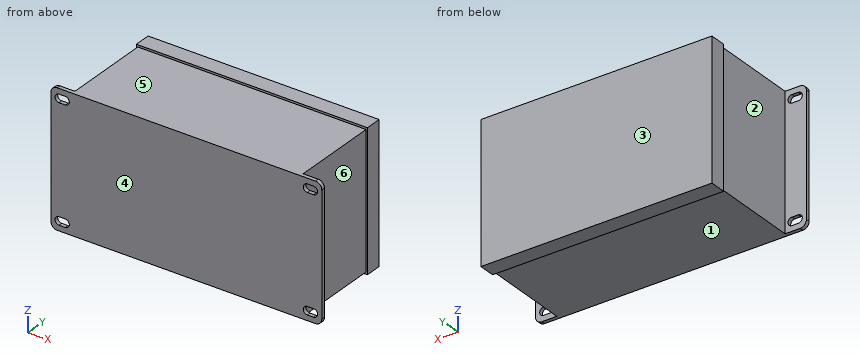
from build123d import *

# Parameters (mm, degrees)
BOSS_EXTRUDE1_DEPTH = 3
SKETCH2_W           = 182
SKETCH2_H           = 107
BOSS_EXTRUDE2_DEPTH = 70
SKETCH4_W           = 184.261814912
SKETCH4_H           = 110.411316032
BOSS_EXTRUDE3_DEPTH = 13


with BuildPart() as part:
    # Sketch1 → Boss-Extrude1 (new body)
    with BuildSketch(Plane(origin=(0, 0, 0), x_dir=(1, 0, 0), z_dir=(0, 1, 0))):
        with BuildLine():
            Line((-103, -53.5), (103, -53.5))
            ThreePointArc((103, -53.5), (106.535533906, -52.035533906), (108, -48.5))
            Line((108, -48.5), (108, 48.5))
            ThreePointArc((108, 48.5), (106.535533906, 52.035533906), (103, 53.5))
            Line((103, 53.5), (-103, 53.5))
            ThreePointArc((-103, 53.5), (-106.535533906, 52.035533906), (-108, 48.5))
            Line((-108, 48.5), (-108, -48.5))
            ThreePointArc((-108, -48.5), (-106.535533906, -52.035533906), (-103, -53.5))
        make_face()
        with BuildLine():
            Line((-101.5, 49.2), (-96.5, 49.2))
            ThreePointArc((-96.5, 49.2), (-93.3, 46), (-96.5, 42.8))
            Line((-96.5, 42.8), (-101.5, 42.8))
            ThreePointArc((-101.5, 42.8), (-104.7, 46), (-101.5, 49.2))
        make_face(mode=Mode.SUBTRACT)
        with BuildLine():
            Line((96.5, 49.2), (101.5, 49.2))
            ThreePointArc((101.5, 49.2), (104.7, 46), (101.5, 42.8))
            Line((101.5, 42.8), (96.5, 42.8))
            ThreePointArc((96.5, 42.8), (93.3, 46), (96.5, 49.2))
        make_face(mode=Mode.SUBTRACT)
        with BuildLine():
            Line((-101.5, -42.8), (-96.5, -42.8))
            ThreePointArc((-96.5, -42.8), (-93.3, -46), (-96.5, -49.2))
            Line((-96.5, -49.2), (-101.5, -49.2))
            ThreePointArc((-101.5, -49.2), (-104.7, -46), (-101.5, -42.8))
        make_face(mode=Mode.SUBTRACT)
        with BuildLine():
            Line((96.5, -42.8), (101.5, -42.8))
            ThreePointArc((101.5, -42.8), (104.7, -46), (101.5, -49.2))
            Line((101.5, -49.2), (96.5, -49.2))
            ThreePointArc((96.5, -49.2), (93.3, -46), (96.5, -42.8))
        make_face(mode=Mode.SUBTRACT)
    extrude(amount=BOSS_EXTRUDE1_DEPTH)

    # Sketch2 → Boss-Extrude2 (add)
    with BuildSketch(Plane(origin=(0, 3, 0), x_dir=(1, 0, 0), z_dir=(0, 1, 0))):
        Rectangle(SKETCH2_W, SKETCH2_H)
    extrude(amount=BOSS_EXTRUDE2_DEPTH)

    # Sketch4 → Boss-Extrude3 (add)
    with BuildSketch(Plane(origin=(0, 73, 0), x_dir=(1, 0, 0), z_dir=(0, 1, 0))):
        Rectangle(SKETCH4_W, SKETCH4_H)
    extrude(amount=BOSS_EXTRUDE3_DEPTH)


solid = part.part
Here's how the part is built. I have some questions about the finished solid (model axes, mm). Face numbers are marked on the shaded views. A direction names the side the tool comes from. Round coordinates to 2 decimals unless told otherwise and drop trailing zeros. Loops run counter-clockwise (first coordinate to the right, second up) from the corner with the lowest first, then second, coordinate; pieces in that order, holes last. Notation, with made-up numbers: (4.5, 37.5) - (62.5, 37.5) arc R19 ccw to (62.5, 50.5) - close; hole circle Ø7 at (33, -17.75). An arc over 180 degrees is marked (long way). One line per question, with ' | ' between items. Start each with the question number.
Q1. We'd pull the mould along Y, two halves only. Please class the marked faces 3, 4, 5 and 6: +Y half, -Y half, draft (parallel to the pull), parting line (faces both ways), or undercut.
Q2. I want a section at A-A (z = -46). Write out the boundary of the cut face in (x, y), then the cut area to 3 significant figures.
Q3. I want a section at D-D (y = 55). Write out the boundary of the cut face in (x, z).
Q4. For the marked faces 1 and 2, which set-ups out of +Z, -Z, +X, -X, +Y, -Y let a thin tool reach every point of the face, with its end or its side?
Q5. I want a section at C-C (x = 49). Write out the boundary of the cut face in (y, z).
Q6. Please list where these lines run through material, in increasing order: line 1 (X direction, y = 15.5, z = -10); line 2 (Z direction, x = -43, y = 52); line 3 (Y direction, x = -96, z = -7). Write a range as [from, to].
Q7. Will these pins go through, and if not, where does the flat tip stop? pin 1 (5 mm diameter, centred on x = 40.5, y = 20.5, fed in from +Z); pin 2 (2 mm diameter, centred on y = 35.5, z = -42.5, fed in from +X); pin 3 (6.5 mm diameter, centred on y = 80.5, z = -3.5, fed in from -X).
Q8. I want a section at B-B (z = -2). Write out the boundary of the cut face in (x, y), then the cut area to 3 significant figures.
Response values:
1) face 3: +Y half | face 4: -Y half | face 5: draft | face 6: undercut
2) outline: (-108, 0) - (-104.7, 0) - (-104.7, 3) - (-108, 3) - close; (-93.3, 0) - (93.3, 0) - (93.3, 3) - (91, 3) - (91, 73) - (92.13, 73) - (92.13, 86) - (-92.13, 86) - (-92.13, 73) - (-91, 73) - (-91, 3) - (-93.3, 3) - close; (104.7, 0) - (108, 0) - (108, 3) - (104.7, 3) - close | area: 15,700 mm²
3) outline: (-91, -53.5) - (91, -53.5) - (91, 53.5) - (-91, 53.5) - close
4) face 1: -Z, +X, -X, -Y | face 2: +Z, -Z, -X
5) outline: (0, -53.5) - (73, -53.5) - (73, -55.21) - (86, -55.21) - (86, 55.21) - (73, 55.21) - (73, 53.5) - (0, 53.5) - close
6) line 1: x = [-91, 91] | line 2: z = [-53.5, 53.5] | line 3: y = [0, 3]
7) pin 1: stops at z = 53.5 | pin 2: stops at x = 91 | pin 3: stops at x = -92.13
8) outline: (-108, 0) - (108, 0) - (108, 3) - (91, 3) - (91, 73) - (92.13, 73) - (92.13, 86) - (-92.13, 86) - (-92.13, 73) - (-91, 73) - (-91, 3) - (-108, 3) - close | area: 15,800 mm²
